Answer from the drawing. Dimensions are ordinates in mm from the lowest x, y and z of the part. Coordinates: 2 decimals unless noted, no trailing zeros. Order: outer loops, then holes, each group sorted by start corner. A loop starts at its lowest first (then second) coordinate and runs counter-clockwise, first axis right, second up. Notation, with made-up numbers: (24.25, 85) -> (47.25, 85) arc R21 cw to (47.25, 96) -> close; hole circle Ø1 at (23.25, 46). An arc over 180 degrees is marked (long way). Use CSV: the item, a comma, the result in double quotes.
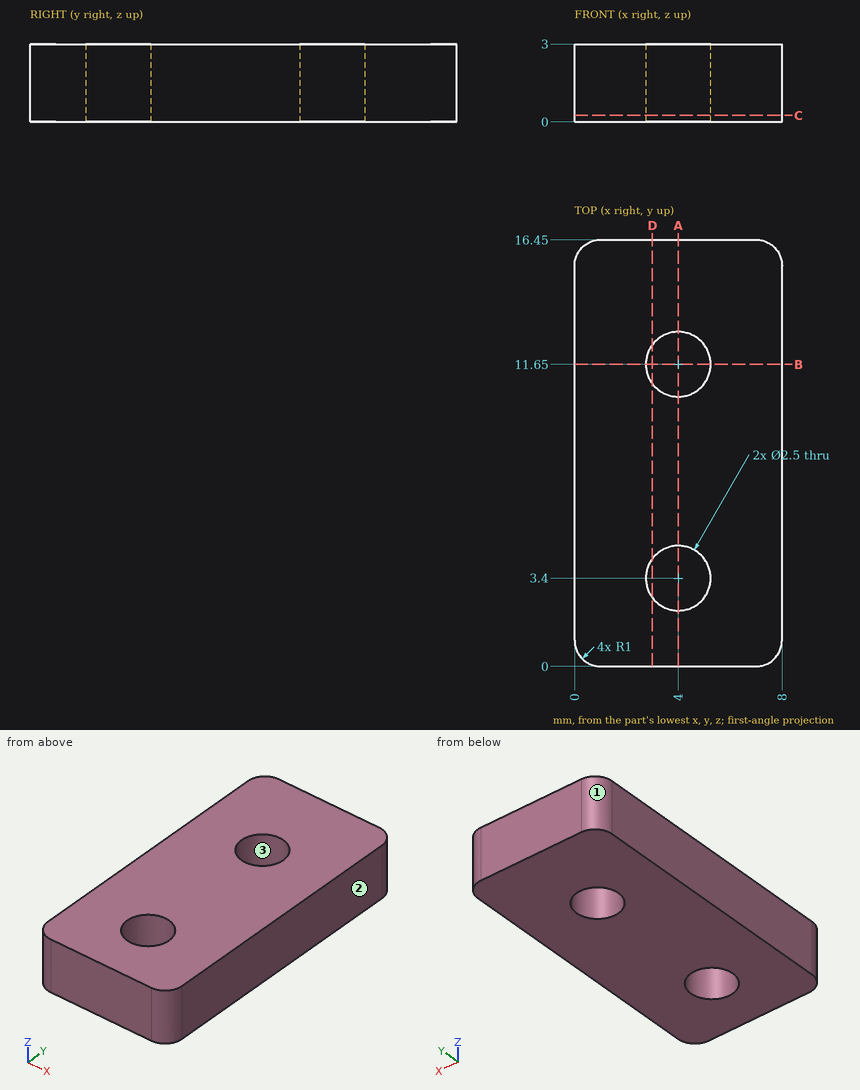
Item 1: Find section D-D, the plane x = 3. Give the vertices of the cut face in (y, z).
Return value:
outline,"(0, 0) -> (2.65, 0) -> (2.65, 3) -> (0, 3) -> close; (4.15, 0) -> (10.9, 0) -> (10.9, 3) -> (4.15, 3) -> close; (12.4, 0) -> (16.45, 0) -> (16.45, 3) -> (12.4, 3) -> close"
Item 2: The mould has two halves that part along X. Classify the marked faces 1, 2 and 3: +X half, -X half, draft (parallel to the pull), parting line (faces both ways), or undercut.
Return value:
face 1,"-X half"
face 2,"+X half"
face 3,"undercut"
Item 3: Find section A-A, the plane x = 4. Give the vertices of the cut face in (y, z).
Return value:
outline,"(0, 0) -> (2.15, 0) -> (2.15, 3) -> (0, 3) -> close; (4.65, 0) -> (10.4, 0) -> (10.4, 3) -> (4.65, 3) -> close; (12.9, 0) -> (16.45, 0) -> (16.45, 3) -> (12.9, 3) -> close"
Item 4: Straight lines are drawn through the part: line 1 along Y through (x, z) = (4, 1.05); line 2 along Y through (x, z) = (3.25, 1.1); line 3 along X through (y, z) = (4.5, 1.55). For each, find the intervals that lie inside material, in ascending order.
Return value:
line 1,"y = 0 to 2.15, 4.65 to 10.4, 12.9 to 16.45"
line 2,"y = 0 to 2.4, 4.4 to 10.65, 12.65 to 16.45"
line 3,"x = 0 to 3.41, 4.59 to 8"
Item 5: Find section B-B, the plane y = 11.65. Give the vertices of the cut face in (x, z), then the cut area to 3 significant figures.
Return value:
outline,"(0, 0) -> (2.75, 0) -> (2.75, 3) -> (0, 3) -> close; (5.25, 0) -> (8, 0) -> (8, 3) -> (5.25, 3) -> close"
area,"16.5 mm^2"
Item 6: Find section C-C, the plane z = 0.25. Give the vertices of the cut face in (x, y).
Return value:
outline,"(0, 1) arc R1 ccw to (1, 0) -> (7, 0) arc R1 ccw to (8, 1) -> (8, 15.45) arc R1 ccw to (7, 16.45) -> (1, 16.45) arc R1 ccw to (0, 15.45) -> close; hole circle Ø2.5 at (4, 3.4); hole circle Ø2.5 at (4, 11.65)"
